```python
from build123d import *

# Parameters (mm, degrees)
SKETCH1_R           = 17.5
BOSS_EXTRUDE1_DEPTH = 790
FILLET1_R           = 50
FILLET3_R           = 50


with BuildPart() as part:
    # Sketch1 → Boss-Extrude1 (new body)
    with BuildSketch(Plane.XY):
        with BuildLine():
            Line((7.791320793, 31.552263315), (145.258384303, -2.393003291))
            Line((145.258384303, -2.393003291), (170.412288606, 46.028262492))
            Line((170.412288606, 46.028262492), (177.818310073, 46.028262492))
            Line((177.818310073, 46.028262492), (150.622769958, -186.130384226))
            Line((150.622769958, -186.130384226), (107.433938335, -20.538722405))
            Line((107.433938335, -20.538722405), (25.187514406, -20.538722405))
            ThreePointArc((25.187514406, -20.538722405), (-30.82642683, -10.294727238), (7.791320793, 31.552263315))
        make_face()
        with Locations(Location((0, 0, 0), (0, 0, 180))):
            Circle(SKETCH1_R, mode=Mode.SUBTRACT)
    extrude(amount=BOSS_EXTRUDE1_DEPTH)

    # Fillet1
    fillet1_edges = [part.edges().sort_by_distance(p)[0] for p in [
        (145.258384303, -2.393003291, 395),
    ]]
    fillet(fillet1_edges, radius=FILLET1_R)

    # Fillet3
    fillet3_edges = [part.edges().sort_by_distance(p)[0] for p in [
        (107.433938335, -20.538722405, 395),
    ]]
    fillet(fillet3_edges, radius=FILLET3_R)


solid = part.part
```
Here's how the part is built. I have some questions about the finished solid (model axes, mm). A direction names the side the tool comes from. Round coordinates to 2 decimals unless told otherwise and drop trailing zeros. Order: outer loops, then holes, each group sorted by start corner. A loop starts at its lowest first (then second) coordinate and runs counter-clockwise, first axis right, second up. Notation, with made-up numbers: M 86.25,30.5 L 112.25,30.5 A32 cw 112.25,63.5 Z; hole C 33,71 d7. An arc over 180 degrees is marked long. Answer in a Markdown table with one row per item.
Item 1: Imagine slicing it at B-B, the plane x = 0. Write out the boundary of the cut face in (y, z).
A:
| item | result |
|---|---|
| outline | M -32.5,0 L -17.5,0 L -17.5,790 L -32.5,790 Z; M 17.5,0 L 32.5,0 L 32.5,790 L 17.5,790 Z |
Item 2: Imagine slicing it at A-A, the plane z = 718. Write out the boundary of the cut face in (x, y), and give its area (3 significant figures).
A:
| item | result |
|---|---|
| outline | M 7.79,31.55 A32.5 ccw long 25.19,-20.54 L 68.8,-20.54 A50 cw 117.18,-57.92 L 150.62,-186.13 L 177.82,46.03 L 170.41,46.03 L 163.4,32.54 A50 cw 107.05,7.04 Z; hole C 0,0 d35 |
| area | 13,200 mm2 |
Item 3: For faces 1 (the face through (56.72, 19.47, 389.47)), 2 (the face through (99.007, -30.693, 400.53)), 3 (the face through (-30.505, -11.211, 389.47)), which set-ups out of +Z, -Z, +X, -X, +Y, -Y let a thin tool reach every point of the face, with its end or its side?
A:
| item | result |
|---|---|
| face 1 | +Z, -Z, +Y |
| face 2 | +Z, -Z, -Y |
| face 3 | +Z, -Z |
Item 4: Imagine slicing it at D-D, the plane x = 98. Write out the boundary of the cut face in (y, z).
A:
| item | result |
|---|---|
| outline | M -29.95,0 L 9.28,0 L 9.28,790 L -29.95,790 Z |
Item 5: If I drill on L1, parallel to Y at x = 0, z = 192; L2, parallel to Y at x = -3, z = 717.5; L3, parallel to X at y = -33, z = 525, over which ranges is the centre line in solid material (lowest first)? Write a range as from..to.
A:
| item | result |
|---|---|
| L1 | y = -32.5..-17.5, 17.5..32.5 |
| L2 | y = -32.36..-17.24, 17.24..32.36 |
| L3 | x = 101.83..168.56 |
Item 6: Thinking about a two-plate mould opening in Y: for faces 4 (the face through (3.794, 17.084, 389.47)), 5 (the face through (139.213, 9.838, 400.53)), 6 (the face through (47, -20.539, 389)), which applies, +Y half, -Y half, draft (parallel to the pull), parting line (faces both ways), or undercut?
A:
| item | result |
|---|---|
| face 4 | undercut |
| face 5 | +Y half |
| face 6 | -Y half |
Item 7: Imagine slicing it at C-C, the plane y = -51. Write out the boundary of the cut face in (x, z), and give its area (3 significant figures).
A:
| item | result |
|---|---|
| outline | M 114.83,0 L 166.45,0 L 166.45,790 L 114.83,790 Z |
| area | 40,800 mm2 |
Item 8: I'm going to push flat-ended pins straight in: pin 1 (2 mm diameter, centred on y = -90, z = 394, fed in from -X); pin 2 (12 mm diameter, centred on y = -112, z = 509, fed in from -X); pin 3 (6 mm diameter, centred on y = -52.5, z = 374, fed in from +X). Where does each tip first touch, or does it pass through?
A:
| item | result |
|---|---|
| pin 1 | stops at x = 125.29 |
| pin 2 | stops at x = 129.72 |
| pin 3 | stops at x = 166.63 |
